```python
from build123d import *

# Parameters (mm, degrees)
BASE_PLATE_SKETCH_W   = 180
BASE_PLATE_SKETCH_H   = 85
BASE_PLATE_DEPTH      = 25
COUNTERBORE_SKETCH_R  = 25
COUNTERBORE_50_DEPTH  = 10
THROUGH_HOLE_SKETCH_R = 10
THROUGH_HOLE_20_DEPTH = 20
BACK_KEY_SKETCH_W     = 10
BACK_KEY_SKETCH_H     = 45
BACK_KEY_DEPTH        = 180
KEY_RELIEF_SKETCH_R   = 10
KEY_RELIEF_CUT_DEPTH  = 103.621878759
UPPER_LUG_SKETCH_R    = 15
UPPER_LUG_DEPTH       = 15
LOWER_START           = -15
LOWER_LUG_SKETCH_R    = 15
LOWER_LUG_DEPTH       = 15
LUG_WEB_SKETCH_W      = 90
LUG_WEB_SKETCH_H      = 55
LUG_WEB_DEPTH         = 25
WEB_CUT_A_DEPTH       = 156
WEB_CUT_B_DEPTH       = 156


with BuildPart() as part:
    # Base Plate Sketch → Base Plate (new body)
    with BuildSketch(Plane.XY):
        Rectangle(BASE_PLATE_SKETCH_W, BASE_PLATE_SKETCH_H)
    extrude(amount=BASE_PLATE_DEPTH)

    # Counterbore Sketch → Counterbore Ø50 (cut)
    with BuildSketch(Plane.XY.offset(25)):
        with Locations((45, 0)):
            Circle(COUNTERBORE_SKETCH_R)
    extrude(amount=-COUNTERBORE_50_DEPTH, mode=Mode.SUBTRACT)

    # Through Hole Sketch → Through Hole Ø20 (cut)
    with BuildSketch(Plane.XY.offset(15)):
        with Locations((45, 0)):
            Circle(THROUGH_HOLE_SKETCH_R)
    extrude(amount=-THROUGH_HOLE_20_DEPTH, mode=Mode.SUBTRACT)

    # Back Key Sketch → Back Key (add, through all)
    with BuildSketch(Plane.ZY.offset(90)):
        with Locations((-5, 0)):
            Rectangle(BACK_KEY_SKETCH_W, BACK_KEY_SKETCH_H)
    extrude(amount=-BACK_KEY_DEPTH)

    # Key Relief Sketch → Key Relief Cut (cut, through all)
    with BuildSketch(Plane.XY):
        with Locations((45, 0)):
            Circle(KEY_RELIEF_SKETCH_R)
    extrude(amount=-KEY_RELIEF_CUT_DEPTH, mode=Mode.SUBTRACT)

    # Upper Lug Sketch → Upper Lug (add)
    with BuildSketch(Plane.XZ.offset(42.5)):
        with BuildLine():
            Line((-68.681371492, 88.01203122), (-90, 25))
            Line((-90, 25), (0, 25))
            Line((0, 25), (-21.318628508, 88.01203122))
            ThreePointArc((-21.318628508, 88.01203122), (-45, 105), (-68.681371492, 88.01203122))
        make_face()
        with Locations(Location((-45, 80, 0), (0, 0, 270))):
            Circle(UPPER_LUG_SKETCH_R, mode=Mode.SUBTRACT)
    extrude(amount=-UPPER_LUG_DEPTH)

    # Lower Lug Sketch → Lower Lug (add)
    with BuildSketch(Plane(origin=(0, 42.5, 0), x_dir=(1, 0, 0), z_dir=(0, 1, 0)).offset(LOWER_START)):
        with BuildLine():
            Line((-90, -25), (-68.681371492, -88.01203122))
            ThreePointArc((-68.681371492, -88.01203122), (-45, -105), (-21.318628508, -88.01203122))
            Line((-21.318628508, -88.01203122), (0, -25))
            Line((0, -25), (-90, -25))
        make_face()
        with Locations(Location((-45, -80, 0), (0, 0, 90))):
            Circle(LOWER_LUG_SKETCH_R, mode=Mode.SUBTRACT)
    extrude(amount=LOWER_LUG_DEPTH)

    # Lug Web Sketch → Lug Web (add)
    with BuildSketch(Plane.XY.offset(25)):
        with Locations((-45, 0)):
            Rectangle(LUG_WEB_SKETCH_W, LUG_WEB_SKETCH_H)
    extrude(amount=LUG_WEB_DEPTH)

    # Web Cut A Sketch → Web Cut A (cut, through all)
    with BuildSketch(Plane(origin=(0, 27.5, 0), x_dir=(1, 0, 0), z_dir=(0, 1, 0))):
        Polygon((0, -25), (-8.458157948, -50), (0, -50), align=None)
    extrude(amount=-WEB_CUT_A_DEPTH, mode=Mode.SUBTRACT)

    # Web Cut B Sketch → Web Cut B (cut, through all)
    with BuildSketch(Plane.XZ.offset(27.5)):
        Polygon((-90, 25), (-81.541842052, 50), (-90, 50), align=None)
    extrude(amount=-WEB_CUT_B_DEPTH, mode=Mode.SUBTRACT)


solid = part.part
```
The listing builds one solid part. Answer for the finished solid, in the listing's coordinates (mm). A direction names the side the tool comes from. Round coordinates to 2 decimals unless told otherwise and drop trailing zeros. Loops run counter-clockwise (first coordinate to the right, second up) from the corner with the lowest first, then second, coordinate; pieces in that order, holes last. Notation, with made-up numbers: (46, -32.5) -> (82, -32.5) arc R13 ccw to (82, -16.5) -> close; hole circle Ø10 at (-9, -26.75). An arc over 180 degrees is marked (long way). Use one line per item in the form item = value.
1. The part is cut by section B-B on y = 0. Determine the outline of the cut face in (x, z).
Answer key:
outline = (-90, -10) -> (35, -10) -> (35, 15) -> (20, 15) -> (20, 25) -> (0, 25) -> (-8.46, 50) -> (-81.54, 50) -> (-90, 25) -> close; (55, -10) -> (90, -10) -> (90, 25) -> (70, 25) -> (70, 15) -> (55, 15) -> close
2. For a pull along Z with two mould halves and no side action, classify faces 1 (the flat face through (-90, -1, 11)), 2 (the cylindrical face through (-32.35, -35.11, 71.94)), 3 (the flat face through (24, -18, 25)) as released by +Z, released by -Z, zero draft, split by the parting line, or undercut.
Answer key:
face_1 = zero draft
face_2 = undercut
face_3 = released by +Z
3. The part is cut by section C-C on z = 83.5. Determine the outline of the cut face in (x, y), and give its area (3 significant figures).
Answer key:
outline = (-70.21, -42.5) -> (-59.59, -42.5) -> (-59.59, -27.5) -> (-70.21, -27.5) -> close; (-70.21, 27.5) -> (-59.59, 27.5) -> (-59.59, 42.5) -> (-70.21, 42.5) -> close; (-30.41, -42.5) -> (-19.79, -42.5) -> (-19.79, -27.5) -> (-30.41, -27.5) -> close; (-30.41, 27.5) -> (-19.79, 27.5) -> (-19.79, 42.5) -> (-30.41, 42.5) -> close
area = 637 mm²
4. The part is cut by section D-D on y = 36. Determine the outline of the cut face in (x, z).
Answer key:
outline = (-90, 0) -> (90, 0) -> (90, 25) -> (0, 25) -> (-21.32, 88.01) arc R25 ccw to (-68.68, 88.01) -> (-90, 25) -> close; hole circle Ø30 at (-45, 80)
5. Flat-ended cylindrical pins translate along their axes: pin 1 Ø8 at (x, z) = (29.5, -6.5) entering from -Y; pin 2 Ø3 at (x, z) = (18.5, -7) entering from +Y; pin 3 Ø2 at (y, z) = (27, 67.5) entering from -X. Find the tip coordinate at first contact, or state that the pin passes through.
Answer key:
pin_1 = -22.5
pin_2 = 22.5
pin_3 = -75.91
6. A tool of negligible diameter and unlimited length cuts with its end or side. For faces 4 (the flat face through (-37, 27.5, 65)), 5 (the flat face through (-1, 22.5, -5)), 6 (the flat face through (-1, -32, 0)), 7 (the cylindrical face through (25, -15, 20)), 8 (the flat face through (-21, 42.5, 40)), from which of +Z, -Z, +X, -X, +Y, -Y can it reach the whole face along a straight path? Write none if from no direction.
Answer key:
face_4 = +Z, +X, -X
face_5 = -Z, +X, -X, +Y
face_6 = -Z, +X, -X, -Y
face_7 = +Z
face_8 = +Z, -Z, +X, -X, +Y
7. Find the intervals of material crossed by probe 1 along Y at (x, z) = (45, -5); probe 2 along Y at (x, z) = (45, 21.25); probe 3 along Z at (x, y) = (11, -29.5), in increasing order. Write a range as [from, to].
Answer key:
probe_1 = [-22.5, -10], [10, 22.5]
probe_2 = [-42.5, -25], [25, 42.5]
probe_3 = [0, 25]
8. The part is cut by section A-A on x = -45. Determine the outline of the cut face in (y, z).
Answer key:
outline = (-42.5, 0) -> (-22.5, 0) -> (-22.5, -10) -> (22.5, -10) -> (22.5, 0) -> (42.5, 0) -> (42.5, 65) -> (27.5, 65) -> (27.5, 50) -> (-27.5, 50) -> (-27.5, 65) -> (-42.5, 65) -> close; (-42.5, 95) -> (-27.5, 95) -> (-27.5, 105) -> (-42.5, 105) -> close; (27.5, 95) -> (42.5, 95) -> (42.5, 105) -> (27.5, 105) -> close
